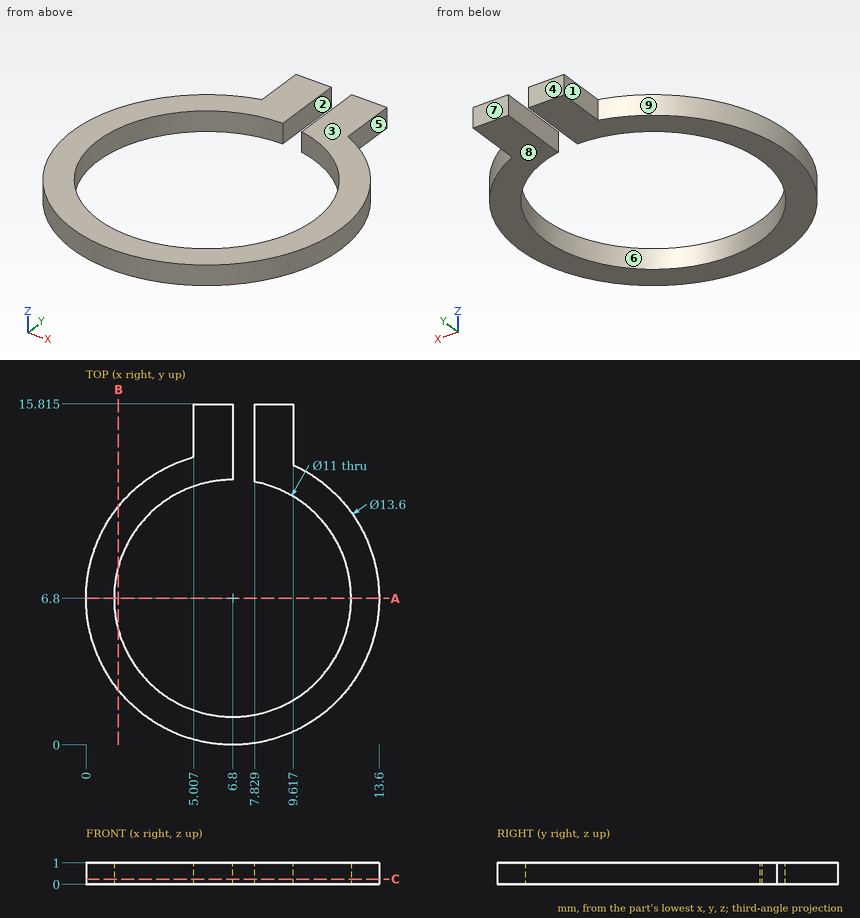
Geometry check sheet. Reference: drawing and pictorial views, mm from the part's lowest x, y, z. A direction names the side the tool comes from. Round coordinates to 2 decimals unless told otherwise and drop trailing zeros. Write each loop counter-clockwise with the first axis right and the second up, starting at its lowest first coordinate (ties: lowest second). Pieces come first, ordered by that corner, then holes.
1. Section check B-B on x = 1.5. Enter the section's corners in (y, z).
2. Access from +Z, -Z, +X, -X, +Y, -Y to the whole of each face (thin tool, end or side, straight path). Record for the marked faces 1, 2, 3, 4 and 5.
3. Section check C-C on z = 0.25. Enter the section's corners in (x, y) (1 decimal), plus the area to 3 significant figures.
4. Gauge pin test, flat end, axial feed: P1, Ø0.5, axis at y = 15, z = 0.5, coming from the -X side. Record the tip position at first contact, or that the pin passes through.
5. Draft check along Y on the marked faces 6, 7, 8 and 9. Enter one of: +Y half, -Y half, draft (parallel to the pull), parting line (faces both ways), or undercut.
6. Scan lines: L1, parallel to X at y = 6.8, z = 0.4; L2, parallel to Y at x = 8.5, z = 0.3 (1 decimal); L3, parallel to Y at x = 11.5, z = 0.65 (1 decimal). Record each from-to range of solid material in increasing order.
7. Section check A-A on y = 6.8. Enter the section's corners in (x, z).
Answer:
1. outline: (2.54, 0) - (5.33, 0) - (5.33, 1) - (2.54, 1) - close; (8.27, 0) - (11.06, 0) - (11.06, 1) - (8.27, 1) - close
2. face 1: +Z, -Z, -X, +Y
2. face 2: +Z, -Z, +Y
2. face 3: +Z, +X, -X, +Y, -Y
2. face 4: +Z, -Z, +X, -X, +Y
2. face 5: +Z, -Z, +X, +Y
3. outline: (5, 13.4) arc R6.8 ccw (long way) to (9.6, 13) - (9.6, 15.8) - (7.8, 15.8) - (7.8, 12.2) arc R5.5 cw (long way) to (6.8, 12.3) - (6.8, 15.8) - (5, 15.8) - close
3. area: 57.5 mm2
4. P1: stops at x = 5.01
5. face 6: undercut
5. face 7: +Y half
5. face 8: draft
5. face 9: parting line
6. L1: x = 0 to 1.3, 12.3 to 13.6
6. L2: y = 0.2 to 1.6, 12 to 15.8
6. L3: y = 1.9 to 3.9, 9.7 to 11.7
7. outline: (0, 0) - (1.3, 0) - (1.3, 1) - (0, 1) - close; (12.3, 0) - (13.6, 0) - (13.6, 1) - (12.3, 1) - close
